```python
from build123d import *

# Parameters (mm, degrees)
BOSS_EXTRUDE1_DEPTH = 8
CUT_EXTRUDE1_DEPTH  = 10
SKETCH3_W           = 4.5
SKETCH3_H           = 30
CUT_EXTRUDE2_DEPTH  = 10


with BuildPart() as part:
    # Sketch1 → Boss-Extrude1 (new body)
    with BuildSketch(Plane.XY):
        with BuildLine():
            Line((-94.65, 0), (98.35, 0))
            ThreePointArc((98.35, 0), (1.85, 96.5), (-94.65, 0))
        make_face()
    extrude(amount=BOSS_EXTRUDE1_DEPTH)

    # Sketch2 → Cut-Extrude1 (cut)
    with BuildSketch(Plane.XY.offset(8)):
        Polygon((-94.65, 0), (-94.65, 25), (109.452328138, 25), (98.649241205, -24.174377991), align=None)
    extrude(amount=-CUT_EXTRUDE1_DEPTH, mode=Mode.SUBTRACT)

    # Sketch3 → Cut-Extrude2 (cut)
    with BuildSketch(Plane(origin=(0, 0, 0), x_dir=(-1, 0, 0), z_dir=(0, 0, -1))):
        with Locations((0, 40)):
            Rectangle(SKETCH3_W, SKETCH3_H)
        with Locations((52.5, 40)):
            Rectangle(SKETCH3_W, SKETCH3_H)
        with Locations((-52.5, 40)):
            Rectangle(SKETCH3_W, SKETCH3_H)
    extrude(amount=-CUT_EXTRUDE2_DEPTH, mode=Mode.SUBTRACT)


solid = part.part
```
Can you work these out from the model? Positions are in its coordinate system, mm. A direction names the side the tool comes from. Round coordinates to 2 decimals unless told otherwise and drop trailing zeros. Loops run counter-clockwise (first coordinate to the right, second up) from the corner with the lowest first, then second, coordinate; pieces in that order, holes last. Notation, with made-up numbers: (54, 84) -> (112, 84) arc R28 cw to (112, 110) -> close; hole circle Ø9 at (44, 69). An arc over 180 degrees is marked (long way). One line per item, written item: value. Start each with the question number.
1. If I drill on probe 1 along X at (y, z) = (48.5, 2.5); probe 2 along X at (y, z) = (45.5, 7.25); probe 3 along Y at (x, z) = (4, 1.5), over which ranges is the centre line in solid material (lowest first)?
2. If we mould it in two halves opening along X, with no side actions, what happens to faces 3 (the flat face through (-27, 25, 4)), 4 (the flat face through (-50.25, 40, 4)), 5 (the cylindrical face through (3.618, 96.484, 3.944)), 6 (the flat face through (-2.25, 40, 4))? For each: pulls with the +X half, pulls with the -X half, needs draft (parallel to the pull), parting line crosses it, or undercut.
3. If we section it at B-B, the plane z = 6.25: Write out the boundary of the cut face in (x, y).
4. For faces 1 (the flat face through (2.25, 40, 4)), 2 (the flat face through (26, 25, 4)), which set-ups out of +Z, -Z, +X, -X, +Y, -Y let a thin tool reach every point of the face, with its end or its side?
5. If we section it at C-C, the plane y = 51.5: Write out the boundary of the cut face in (x, z), then the cut area to 3 significant figures.
6. If we section it at D-D, the plane x = -22: Write out the boundary of the cut face in (y, z).
7. For pin 1 (2.5 mm diameter, centred on y = 45.5, z = 3, fed in from +X); pin 2 (4 mm diameter, centred on y = 34, z = 2.5, fed in from +X); pin 3 (4 mm diameter, centred on y = 45.5, z = 4.5, fed in from -X), each with a flat end and sliding along its axis, tell me the tip position at first contact or that it passes through.
8. If we section it at A-A, the plane y = 40.5: Write out the boundary of the cut face in (x, z).
Calculated:
1. probe 1: x = -81.58 to -54.75, -50.25 to -2.25, 2.25 to 50.25, 54.75 to 85.28
1. probe 2: x = -83.25 to -54.75, -50.25 to -2.25, 2.25 to 50.25, 54.75 to 86.95
1. probe 3: y = 25 to 96.48
2. face 3: needs draft
2. face 4: undercut
2. face 5: parting line crosses it
2. face 6: undercut
3. outline: (-91.36, 25) -> (-54.75, 25) -> (-54.75, 55) -> (-50.25, 55) -> (-50.25, 25) -> (-2.25, 25) -> (-2.25, 55) -> (2.25, 55) -> (2.25, 25) -> (50.25, 25) -> (50.25, 55) -> (54.75, 55) -> (54.75, 25) -> (95.06, 25) arc R96.5 ccw to start
4. face 1: +Z, -Z, -Y
4. face 2: +Z, -Z, +X, -X, -Y
5. outline: (-79.76, 0) -> (-54.75, 0) -> (-54.75, 8) -> (-79.76, 8) -> close; (-50.25, 0) -> (-2.25, 0) -> (-2.25, 8) -> (-50.25, 8) -> close; (2.25, 0) -> (50.25, 0) -> (50.25, 8) -> (2.25, 8) -> close; (54.75, 0) -> (83.46, 0) -> (83.46, 8) -> (54.75, 8) -> close
5. area: 1,200 mm²
6. outline: (25, 0) -> (93.51, 0) -> (93.51, 8) -> (25, 8) -> close
7. pin 1: stops at x = 87.61
7. pin 2: stops at x = 92.89
7. pin 3: stops at x = -84.29
8. outline: (-85.74, 0) -> (-54.75, 0) -> (-54.75, 8) -> (-85.74, 8) -> close; (-50.25, 0) -> (-2.25, 0) -> (-2.25, 8) -> (-50.25, 8) -> close; (2.25, 0) -> (50.25, 0) -> (50.25, 8) -> (2.25, 8) -> close; (54.75, 0) -> (89.44, 0) -> (89.44, 8) -> (54.75, 8) -> close
